Verification items for the finished model (mm, model axes). Face numbers are marked on the shaded views. Round coordinates to 2 decimals unless told otherwise and drop trailing zeros. Loops run counter-clockwise (first coordinate to the right, second up) from the corner with the lowest first, then second, coordinate; pieces in that order, holes last. Notation, with made-up numbers: M 40.25,0.5 L 45.25,0.5 A14 cw 45.25,16.5 Z; hole C 17,26 d9. An arc over 180 degrees is marked long. One line per item, written item: value.
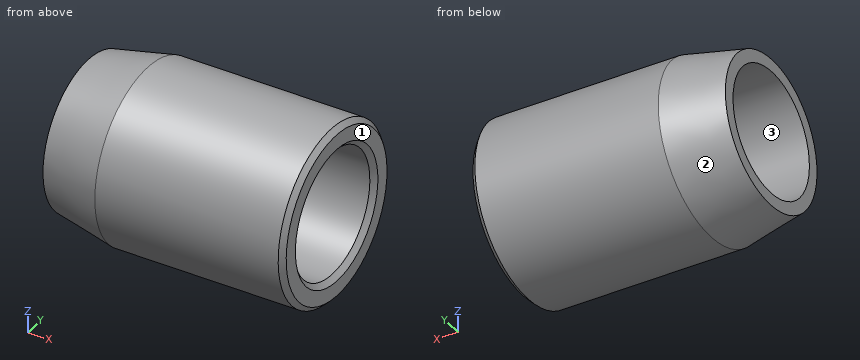
from build123d import *

# Parameters (mm, degrees)
CHAMFER1_SIZE = 1


with BuildPart() as part:
    # Sketch1 → Revolve1 (revolve)
    with BuildSketch(Plane.XY, mode=Mode.PRIVATE) as revolve1_sk:
        Polygon((0, 12.5), (0, 17.5), (-38, 17.5), (-50, 15), (-50, 12.5), align=None)
    revolve(revolve1_sk.sketch.rotate(Axis((0, 0, 0), (-1, 0, 0)), 90), axis=Axis((0, 0, 0), (-1, 0, 0)))

    # Chamfer1
    chamfer1_edges = [part.edges().sort_by_distance(p)[0] for p in [
        (0, 0, 17.5),
        (0, 0, 12.5),
    ]]
    chamfer(chamfer1_edges, length=CHAMFER1_SIZE)


solid = part.part
(1) Mould release check, pull along Y, two halves, no side actions. Record for the marked faces 1, 2 and 3: +Y half, -Y half, draft (parallel to the pull), parting line (faces both ways), or undercut.
Completed:
face 1: draft
face 2: parting line
face 3: undercut
(2) Sectioned sample at C-C on x = -6.5. Enter the section's corners in (y, z), and give its area (3 significant figures).
Completed:
outline: C 0,0 d35; hole C 0,0 d25
area: 471 mm^2
(3) Sectioned sample at D-D on x = -45.5. Enter the section's corners in (y, z) (1 decimal).
Completed:
outline: C 0,0 d31.9; hole C 0,0 d25
(4) Thickness scan on L1, parallel to Y at x = -25, z = 0; L2, parallel to Y at x = -40, z = 0; L3, parallel to Z at x = -44.5, y = -8.5. Record the ranges inside material, lowest first. Write a range as from..to.
Completed:
L1: y = -17.5..-12.5, 12.5..17.5
L2: y = -17.08..-12.5, 12.5..17.08
L3: z = -13.73..-9.17, 9.17..13.73
(5) Depth check by flat-ended pin: pin 1 Ø1 at (x, z) = (-26.5, 5) entering from +Y; pin 2 Ø1.5 at (x, z) = (-7.5, 13.5) entering from +Y. Enter the tip coordinate at first touch or a pass-through.
Completed:
pin 1: stops at y = 16.91
pin 2: stops at y = 11.99
(6) Sectioned sample at A-A on y = 0. Enter the section's corners in (x, z).
Completed:
outline: M -50,-15 L -38,-17.5 L -1,-17.5 L 0,-16.5 L 0,-13.5 L -1,-12.5 L -50,-12.5 Z; M -50,12.5 L -1,12.5 L 0,13.5 L 0,16.5 L -1,17.5 L -38,17.5 L -50,15 Z
